Model file for the job. Use its own axes, mm. A direction names the side the tool comes from. Give positions to 0.01 mm unless a question says otherwise; leave off trailing zeros. Write each loop counter-clockwise with the first axis right and the second up, starting at its lowest first coordinate (ties: lowest second). Pieces come first, ordered by that corner, then holes. Notation, with made-up numbers: M 42.25,-8.5 L 94.25,-8.5 A33 ccw 94.25,21.5 Z; hole C 44.5,16.25 d2. An arc over 180 degrees is marked long. Answer as a JSON object with one key per item and string values. Group by question number.
```python
from build123d import *

# Parameters (mm, degrees)
CHAMFER1_SIZE = 0.5


with BuildPart() as part:
    # Sketch1 → Revolve1 (revolve)
    with BuildSketch(Plane(origin=(0, 0, 0), x_dir=(0, 0, -1), z_dir=(1, 0, 0)), mode=Mode.PRIVATE) as revolve1_sk:
        Polygon((0, 0), (7.5, 0), (7.5, -5), (5, -5), (5, -55), (2.425, -55), (2.425, -60), (0, -60), align=None)
    revolve(revolve1_sk.sketch.rotate(Axis((0, 0, 0), (0, -1, 0)), 180), axis=Axis((0, 0, 0), (0, -1, 0)))

    # Chamfer1
    chamfer1_edges = [part.edges().sort_by_distance(p)[0] for p in [
        (0, -60, -2.425),
        (0, -55, -5),
        (0, -5, -7.5),
        (0, 0, -7.5),
    ]]
    chamfer(chamfer1_edges, length=CHAMFER1_SIZE)


solid = part.part
```
Q1. Slice it at C-C, the plane y = -12.5. Write the cut outline in (x, z).
Q2. Slice it at B-B, the plane z = 0. Write the cut outline in (x, y) (3 decimals).
Q3. Slice it at A-A, the plane x = 0. Write the cut outline in (y, z) (3 decimals).
Q4. Wall check: L1, parallel to Y at x = 5.5, z = 1; L2, parallel to Y at x = -1.5, z = -3; L3, parallel to X at y = -2.5, z = -6. Give the ranges that are in metal, low to high.
Q5. 3-axis set-ups, long thin cutter, end or side, ignore diameter. For faces 1 (the flat face through (0, 0, 0)), 2 (the flat face through (-5, -5, -2)): which of +Z, -Z, +X, -X, +Y, -Y reach the whole face in a straight line?
Q6. Drop flat-ended pins along their axis: P1, Ø3, axis at x = -5.5, y = -43, coming from the -Z side; P2, Ø8, axis at y = -30.5, z = 0.5, coming from the +X side. Give the stop position or say it passes through.
Solved:
{
 "1": {"outline": "C 0,0 d10"},
 "2": {"outline": "M -7.5,-4.5 L -7,-5 L -5,-5 L -5,-54.5 L -4.5,-55 L -2.425,-55 L -2.425,-59.5 L -1.925,-60 L 1.925,-60 L 2.425,-59.5 L 2.425,-55 L 4.5,-55 L 5,-54.5 L 5,-5 L 7,-5 L 7.5,-4.5 L 7.5,-0.5 L 7,0 L -7,0 L -7.5,-0.5 Z"},
 "3": {"outline": "M -60,-1.925 L -59.5,-2.425 L -55,-2.425 L -55,-4.5 L -54.5,-5 L -5,-5 L -5,-7 L -4.5,-7.5 L -0.5,-7.5 L 0,-7 L 0,7 L -0.5,7.5 L -4.5,7.5 L -5,7 L -5,5 L -54.5,5 L -55,4.5 L -55,2.425 L -59.5,2.425 L -60,1.925 Z"},
 "4": {"L1": "y = -5 to 0", "L2": "y = -55 to 0", "L3": "x = -4.5 to 4.5"},
 "5": {"face 1": "+Z, -Z, +X, -X, +Y", "face 2": "-Y"},
 "6": {"P1": "stops at z = -3", "P2": "stops at x = 5"}
}
